Here's how the part is built. I have some questions about the finished solid (model axes, mm). Face numbers are marked on the shaded views. A direction names the side the tool comes from. Round coordinates to 2 decimals unless told otherwise and drop trailing zeros. Order: outer loops, then holes, each group sorted by start corner. A loop starts at its lowest first (then second) coordinate and runs counter-clockwise, first axis right, second up. Notation, with made-up numbers: (-9.5, 4.5) - (43.5, 4.5) arc R19 ccw to (43.5, 21.5) - close; hole circle Ø9 at (-29, -25.75). An arc over 180 degrees is marked (long way). One line per item, written item: value.
from build123d import *

# Parameters (mm, degrees)
CHAMFER1_SIZE = 0.5


with BuildPart() as part:
    # Sketch1 → Revolve1 (revolve)
    with BuildSketch(Plane(origin=(0, 0, 0), x_dir=(0, 0, -1), z_dir=(1, 0, 0))):
        Polygon((0, 15), (5.25, 15), (5.25, 5), (7.5, 5), (7.5, 0), (0, 0), align=None)
    revolve(axis=Axis((0, 0, 0), (0, 1, 0)))

    # Chamfer1
    chamfer1_edges = [part.edges().sort_by_distance(p)[0] for p in [
        (0, 0, 7.5),
        (0, 5, 7.5),
        (0, 15, 5.25),
    ]]
    chamfer(chamfer1_edges, length=CHAMFER1_SIZE)


solid = part.part
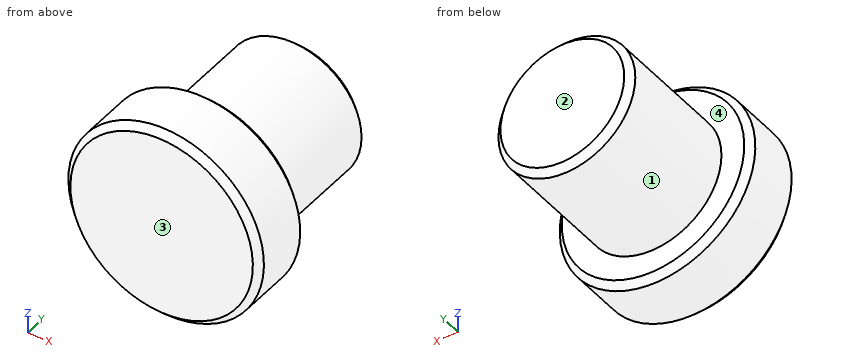
Q1. If we section it at B-B, the plane x = 0: Please give me the cut outline in (y, z), then the cut area to 3 significant figures.
Results list:
outline: (0, -7) - (0.5, -7.5) - (4.5, -7.5) - (5, -7) - (5, -5.25) - (14.5, -5.25) - (15, -4.75) - (15, 4.75) - (14.5, 5.25) - (5, 5.25) - (5, 7) - (4.5, 7.5) - (0.5, 7.5) - (0, 7) - close
area: 179 mm²
Q2. Which directions (+Z, -Z, +X, -X, +Y, -Y) give clear straight access to the entire face, cutting with the end or side of a thin tool? Please do the marked faces 3 and 4.
Results list:
face 3: +Z, -Z, +X, -X, -Y
face 4: +Y
Q3. Will these pins go through, and if not, where does the flat tip stop? pin 1 (2 mm diameter, centred on x = 0.5, y = 13.5, fed in from -Z); pin 2 (8 mm diameter, centred on y = 2.5, z = 3.5, fed in from -X); pin 3 (2 mm diameter, centred on x = 5, y = 9.5, fed in from -Z); pin 4 (3 mm diameter, centred on y = 9.5, z = -4, fed in from +X).
Results list:
pin 1: z = -5.25
pin 2: x = -7.5
pin 3: z = -3.4
pin 4: x = 4.62
Q4. If we section it at C-C, the plane y = 3.25: Please give me the cut outline in (x, z), then the cut area to 3 significant figures.
Results list:
outline: circle Ø15 at (0, 0)
area: 177 mm²
Q5. If we section it at A-A, the plane z = 0: Please give me the cut outline in (x, y), then the cut area to 3 significant figures.
Results list:
outline: (-7.5, 0.5) - (-7, 0) - (7, 0) - (7.5, 0.5) - (7.5, 4.5) - (7, 5) - (5.25, 5) - (5.25, 14.5) - (4.75, 15) - (-4.75, 15) - (-5.25, 14.5) - (-5.25, 5) - (-7, 5) - (-7.5, 4.5) - close
area: 179 mm²
Q6. We'd pull the mould along Z, two halves only. Please class the marked faces 1 and 2: released by +Z, released by -Z, zero draft, split by the parting line, or undercut.
Results list:
face 1: split by the parting line
face 2: zero draft
Q7. If we section it at D-D, the plane y = 6: Please give me the cut outline in (x, z).
Results list:
outline: circle Ø10.5 at (0, 0)
Q8. If I drill on line 1 along Y through (x, z) = (-2.5, 6.5); line 2 along X through (y, z) = (13.75, 0.25); line 3 along X through (y, z) = (11.5, 3.5), over which ranges is the centre line in solid material (lowest first)?
Results list:
line 1: 0 to 5
line 2: -5.24 to 5.24
line 3: -3.91 to 3.91
